```python
from build123d import *

# Parameters (mm, degrees)
FILLET1_R   = 0.2
FILLET2_R   = 0.25
HEX_2_DEPTH = 2.5


with BuildPart() as part:
    # BodySke → Base-Revolve (revolve)
    with BuildSketch(Plane.XY, mode=Mode.PRIVATE) as base_revolve_sk:
        Polygon((0, 0), (0, 4.25), (5, 4.25), (5, 2.5), (20.555, 2.5), (21, 2.055), (21, 0), align=None)
    revolve(base_revolve_sk.sketch.rotate(Axis((-31.75, 0, 0), (1, 0, 0)), 90), axis=Axis((-31.75, 0, 0), (1, 0, 0)))

    # Fillet1
    fillet1_edges = [part.edges().sort_by_distance(p)[0] for p in [
        (5, 0, -2.5),
    ]]
    fillet(fillet1_edges, radius=FILLET1_R)

    # Fillet2
    fillet2_edges = [part.edges().sort_by_distance(p)[0] for p in [
        (0, 0, -4.25),
    ]]
    fillet(fillet2_edges, radius=FILLET2_R)

    # Sketch2 → Hex-PreBroach (revolve, cut)
    with BuildSketch(Plane.XY, mode=Mode.PRIVATE) as hex_prebroach_sk:
        Polygon((0, 2.042), (2.5, 2.042), (3.67894925, 0), (0, 0), align=None)
    revolve(hex_prebroach_sk.sketch.rotate(Axis((0, 0, 0), (1, 0, 0)), 90), axis=Axis((0, 0, 0), (1, 0, 0)), mode=Mode.SUBTRACT)

    # Sketch3 → Hex 2 (cut)
    with BuildSketch(Plane(origin=(0, 0, 0), x_dir=(0, 0.500000000000001, 0.866025403784438), z_dir=(-1, 0, 0))):
        Polygon((1.17894925, 2.042), (-1.17894925, 2.042), (-2.357898499, 0), (-1.17894925, -2.042), (1.17894925, -2.042), (2.357898499, 0), align=None)
    extrude(amount=-HEX_2_DEPTH, mode=Mode.SUBTRACT)


solid = part.part
```
Geometry: final body of the model. Coordinates: model frame, mm. A direction names the side the tool comes from. Coordinates: 2 decimals unless noted, no trailing zeros. Order: outer loops, then holes, each group sorted by start corner. A loop starts at its lowest first (then second) coordinate and runs counter-clockwise, first axis right, second up. Notation, with made-up numbers: (-33.5, -32.5) -> (-2.5, -32.5) arc R20 ccw to (-2.5, -20.5) -> close; hole circle Ø8 at (27, 25). An arc over 180 degrees is marked (long way). Write item = value, one per line.
(1) Line query: line 1 (X direction, y = 3.25, z = 0.25); line 2 (X direction, y = -1, z = -1.75); line 3 (Z direction, x = 3, y = -3.5). Output: solid intervals per line, ascending.
Solved:
line_1 = 0 to 5
line_2 = 2.52 to 21
line_3 = -2.41 to 2.41
(2) Cut plane A-A on x = 11.25. Return loops of the section in (y, z).
Solved:
outline = circle Ø5 at (0, 0)
(3) Pin query (flat end, axial travel): pin 1 Ø0.7 at (x, y) = (2, -0.5) entering from +Z; pin 2 Ø1.5 at (y, z) = (-0.5, 3) entering from +X; pin 3 Ø0.5 at (y, z) = (0.5, 1.5) entering from -X. Return the tip coordinate at first contact, or that it passes through.
Solved:
pin_1 = 4.25
pin_2 = 20.76
pin_3 = 2.62
(4) Access query for faces 1 (the flat face through (1.232, 1.76, 1.035)), 2 (the flat face through (0, -2, 1)), 3 (the cylindrical face through (13, -0.1, -2.5)). Directions: +Z, -Z, +X, -X, +Y, -Y. A direction counts if a zero-diameter tool reaches every point of the face in a straight line with its end or side. Return the directions, or none.
Solved:
face_1 = -X
face_2 = +Z, -Z, -X, +Y, -Y
face_3 = +X
(5) Cut plane B-B on x = 4.75. Return loops of the section in (y, z), plus the area to 3 significant figures.
Solved:
outline = circle Ø8.5 at (0, 0)
area = 56.7 mm²
(6) Pull-direction query (Z, two-part tool) for faces 4 (the flat face through (21, 0, 0)), 5 (the flat face through (1, 0, 2.042)), 6 (the cylindrical face through (2.658, -4.214, -0.553)); classes: pulls with the +Z half, pulls with the -Z half, needs draft (parallel to the pull), parting line crosses it, or undercut.
Solved:
face_4 = needs draft
face_5 = undercut
face_6 = parting line crosses it
